```python
from build123d import *

# Parameters (mm, degrees)
SKETCH1_R             = 17.5
BOSS_EXTRUDE1_DEPTH   = 6
CHAMFER1_SIZE         = 10
M6_TAPPED_HOLE1_D     = 5
M6_TAPPED_HOLE1_DEPTH = 17
M6_TAPPED_HOLE1_TIP   = 1.502151548
SKETCH8_R             = 2
CUT_EXTRUDE1_DEPTH    = 15
CHAMFER2_SIZE         = 1
M3_TAPPED_HOLE1_D     = 2.5
CHAMFER3_SIZE         = 0.5


with BuildPart() as part:
    # Sketch1 → Boss-Extrude1 (new, symmetric)
    with BuildSketch(Plane(origin=(0, 0, 0), x_dir=(0, 0, -1), z_dir=(1, 0, 0))):
        with BuildLine():
            Line((-36.5, 0), (-10, 0))
            Line((-10, 0), (-10, 10))
            ThreePointArc((-10, 10), (-8.535533906, 13.535533906), (-5, 15))
            Line((-5, 15), (5, 15))
            ThreePointArc((5, 15), (8.535533906, 13.535533906), (10, 10))
            Line((10, 10), (10, 0))
            Line((10, 0), (36.5, 0))
            Line((36.5, 0), (36.5, 85))
            Line((36.5, 85), (-36.5, 85))
            Line((-36.5, 85), (-36.5, 0))
        make_face()
        with Locations((0, 54)):
            Circle(SKETCH1_R, mode=Mode.SUBTRACT)
    extrude(amount=BOSS_EXTRUDE1_DEPTH, both=True)

    # Chamfer1
    chamfer1_edges = [part.edges().sort_by_distance(p)[0] for p in [
        (0, 85, 36.5),
        (0, 85, -36.5),
    ]]
    chamfer(chamfer1_edges, length=CHAMFER1_SIZE)

    # M6 Tapped Hole1
    with Locations(Plane(origin=(0, 0, 0), x_dir=(-1, 0, 0), z_dir=(0, -1, 0))):
        with Locations((0, -25), (0, 25)):
            Hole(M6_TAPPED_HOLE1_D / 2, depth=M6_TAPPED_HOLE1_DEPTH)
            with Locations((0, 0, -(M6_TAPPED_HOLE1_DEPTH + M6_TAPPED_HOLE1_TIP / 2))):  # 118° drill point
                Cone(0, M6_TAPPED_HOLE1_D / 2, M6_TAPPED_HOLE1_TIP, mode=Mode.SUBTRACT)

    # Sketch8 → Cut-Extrude1 (cut)
    with BuildSketch(Plane.XZ):
        with Locations(Location((0, -15, 0), (0, 0, 270))):
            Circle(SKETCH8_R)
        with BuildLine():
            Line((2, 15.5), (2, 14.5))
            ThreePointArc((2, 14.5), (0, 12.5), (-2, 14.5))
            Line((-2, 14.5), (-2, 15.5))
            ThreePointArc((-2, 15.5), (0, 17.5), (2, 15.5))
        make_face()
    extrude(amount=-CUT_EXTRUDE1_DEPTH, mode=Mode.SUBTRACT)

    # Chamfer2
    chamfer2_edges = [part.edges().sort_by_distance(p)[0] for p in [
        (0, 0, -10),
        (0, 0, 10),
    ]]
    chamfer(chamfer2_edges, length=CHAMFER2_SIZE)

    # M3 Tapped Hole1 (through all)
    with Locations(Plane.ZY.offset(6)):
        with Locations((33.5, 44), (33.5, 64), (-16.617009358, 23.240855018), (-30.759144982, 37.382990642), (-33.177357847, 65.023290175), (-21.70582912, 81.406331061)):
            Hole(M3_TAPPED_HOLE1_D / 2)

    # Chamfer3
    chamfer3_edges = [part.edges().sort_by_distance(p)[0] for p in [
        (-6, 54, 17.5),
        (6, 54, 17.5),
    ]]
    chamfer(chamfer3_edges, length=CHAMFER3_SIZE)


solid = part.part
```
Here's how the part is built. I have some questions about the finished solid (model axes, mm). A direction names the side the tool comes from. Give positions to 0.01 mm unless a question says otherwise; leave off trailing zeros. Loops run counter-clockwise (first coordinate to the right, second up) from the corner with the lowest first, then second, coordinate; pieces in that order, holes last. Notation, with made-up numbers: M -34,41.25 L -9,41.25 A5 ccw -9,45.25 Z; hole C 0,-33.75 d1. An arc over 180 degrees is marked long. Use one line per item in the form item = value. Start each with the question number.
Q1. Which directions (+Z, -Z, +X, -X, +Y, -Y) give clear straight access to the entire face, cutting with the end or side of a thin tool? Please do faces 1 (the flat face through (0, 15, 15)), 2 (the flat face through (0, 85, 0)), 3 (the cylindrical face through (0, 13, 9)).
Q2. Will these pins go through, and if not, where does the flat tip stop? pin 1 Ø4.5 at (x, z) = (0, -14.5) entering from -Y; pin 2 Ø2 at (y, z) = (65.02, -33.18) entering from +X; pin 3 Ø5 at (x, z) = (-1.5, 2) entering from -Y; pin 4 Ø4 at (x, z) = (0, 25) entering from -Y.
Q3. If we section it at B-B (z = 33.5): Write out the boundary of the cut face in (x, y).
Q4. If we section it at A-A (y = 5): Write out the boundary of the cut face in (x, z), then the cut area to 3 significant figures.
Q5. If we section it at C-C (z = 0): Write out the boundary of the cut face in (x, y), then the cut area to 4 significant figures.
Q6. If we section it at D-D (x = 4): Write out the boundary of the cut face in (y, z).
Q7. I need wall thicknesses on line 1 along Y through (x, z) = (-2, 33.5); line 2 along Z through (x, y) = (-4.5, 45); line 3 along Z through (x, y) = (-1, 8). Which ranges of each line are inside material? Lowest first, please.
Q8. Thinking about a two-plate mould opening in X: for faces 4 (the cylindrical face through (0.08, 45.24, 33.66)), 5 (the flat face through (0, 15, -15)), 6 (the flat face through (-6, 34, 1)), 7 (the cylindrical face through (-0.33, 8.62, 22.52)), which applies, +X half, -X half, draft (parallel to the pull), parting line (faces both ways), or undercut?
Taken from the geometry:
q1.face_1 = -Y
q1.face_2 = +Z, -Z, +X, -X, +Y
q1.face_3 = +X, -X, -Y
q2.pin_1 = 0
q2.pin_2 = through
q2.pin_3 = 15
q2.pin_4 = 17.3
q3.outline = M -6,0 L 6,0 L 6,42.75 L -6,42.75 Z; M -6,45.25 L 6,45.25 L 6,62.75 L -6,62.75 Z; M -6,65.25 L 6,65.25 L 6,78 L -6,78 Z
q4.outline = M -6,-36.5 L 6,-36.5 L 6,-10 L -6,-10 Z; M -6,10 L 6,10 L 6,36.5 L -6,36.5 Z; hole C 0,-25 d5; hole C 0,25 d5; hole C 0,-15 d4; hole M -2,14.5 A2 ccw 2,14.5 L 2,15.5 A2 ccw -2,15.5 Z
q4.area = 568 mm^2
q5.outline = M -6,15 L 6,15 L 6,36 L 5.5,36.5 L -5.5,36.5 L -6,36 Z; M -6,72 L -5.5,71.5 L 5.5,71.5 L 6,72 L 6,85 L -6,85 Z
q5.area = 419.5 mm^2
q6.outline = M 0,-36.5 L 75,-36.5 L 85,-26.5 L 85,26.5 L 75,36.5 L 0,36.5 L 0,11 L 1,10 L 10,10 A5 cw 15,5 L 15,-5 A5 cw 10,-10 L 1,-10 L 0,-11 Z; hole C 23.24,-16.62 d2.5; hole C 37.38,-30.76 d2.5; hole C 54,0 d35; hole C 44,33.5 d2.5; hole C 64,33.5 d2.5; hole C 65.02,-33.18 d2.5; hole C 81.41,-21.71 d2.5
q7.line_1 = 0 to 42.75, 45.25 to 62.75, 65.25 to 78
q7.line_2 = -36.5 to -15.01, 15.01 to 32.75, 34.25 to 36.5
q7.line_3 = -36.5 to -27.29, -22.71 to -16.73, -13.27 to -10, 10 to 12.77, 17.23 to 22.71, 27.29 to 36.5
q8.face_4 = draft
q8.face_5 = undercut
q8.face_6 = -X half
q8.face_7 = undercut
